The model under review builds one solid part; all positions refer to its coordinate system, in mm. Coordinates: 2 decimals unless noted, no trailing zeros. Order: outer loops, then holes, each group sorted by start corner. A loop starts at its lowest first (then second) coordinate and runs counter-clockwise, first axis right, second up. Notation, with made-up numbers: (75.5, -37) -> (118.5, -37) arc R15 cw to (118.5, -15) -> close; hole circle Ø6 at (-26.5, -36.5). An arc over 180 degrees is marked (long way). Put each result on its own line as item: value.
from build123d import *

# Parameters (mm, degrees)
SKETCH_1_R          = 4
EXTRUDE_1_DEPTH     = 105
CUT_EXTRUDE_1_DEPTH = 10
CUT_EXTRUDE_2_DEPTH = 59


with BuildPart() as part:
    # 草图1 → 凸台-拉伸1 (new body)
    with BuildSketch(Plane.XY):
        with Locations((-9.495904584, 0)):
            Circle(SKETCH_1_R)
    extrude(amount=EXTRUDE_1_DEPTH)

    # 草图2 → 切除-拉伸1 (cut)
    with BuildSketch(Plane(origin=(0, 0, 0), x_dir=(-1, 0, 0), z_dir=(0, 0, -1))):
        with BuildLine():
            Line((7.095904584, 3.2), (11.895904584, 3.2))
            ThreePointArc((11.895904584, 3.2), (9.495904584, 4), (7.095904584, 3.2))
        make_face()
    extrude(amount=-CUT_EXTRUDE_1_DEPTH, mode=Mode.SUBTRACT)

    # 草图3 → 切除-拉伸2 (cut)
    with BuildSketch(Plane(origin=(0, 0, 16), x_dir=(-1, 0, 0), z_dir=(0, 0, -1))):
        with BuildLine():
            Line((7.095904584, 3.2), (11.895904584, 3.2))
            ThreePointArc((11.895904584, 3.2), (9.495904584, 4), (7.095904584, 3.2))
        make_face()
    extrude(amount=-CUT_EXTRUDE_2_DEPTH, mode=Mode.SUBTRACT)


solid = part.part
Item 1: Consider section D-D on z = 85. Write out the cut boundary in (x, y).
Answers below:
outline: circle Ø8 at (-9.5, 0)
Item 2: Consider section B-B on z = 43. Write out the cut boundary in (x, y).
Answers below:
outline: (-11.9, 3.2) arc R4 ccw (long way) to (-7.1, 3.2) -> close
Item 3: For line 1 (Z direction, x = -11.75, y = 3.25); line 2 (X direction, y = 0.25, z = 72.5); line 3 (X direction, y = -3.5, z = 90.5), list the stretches that pass through material, from the lowest coordinate up. Write a range as from..to.
Answers below:
line 1: 10..16, 75..105
line 2: -13.49..-5.5
line 3: -11.43..-7.56
Item 4: Consider section A-A on x = -10.75. Write out the cut boundary in (y, z).
Answers below:
outline: (-3.8, 0) -> (3.2, 0) -> (3.2, 10) -> (3.8, 10) -> (3.8, 16) -> (3.2, 16) -> (3.2, 75) -> (3.8, 75) -> (3.8, 105) -> (-3.8, 105) -> close
Item 5: Consider section C-C on y = 1.75. Write out the cut boundary in (x, z).
Answers below:
outline: (-13.09, 0) -> (-5.9, 0) -> (-5.9, 105) -> (-13.09, 105) -> close
Item 6: Mouldability with a two-part tool opening along Z and no side actions: class faces 1 (the flat face through (-9, 3.2, 45)), 2 (the flat face through (-10, 0, 0)), 3 (the flat face through (-9, 3.2, 5)) as +Z half, -Z half, draft (parallel to the pull), parting line (faces both ways), or undercut.
Answers below:
face 1: undercut
face 2: -Z half
face 3: draft
Item 7: For pin 1 Ø1.5 at (x, y) = (-12, 1.5) entering from -Z; pin 2 Ø2 at (y, z) = (3, 73) entering from -X; pin 3 Ø2.5 at (x, z) = (-9, 5.5) entering from +Y; pin 4 Ø3 at (y, z) = (2.5, 11) entering from +X, all flat-tipped, find the tip position at first contact; note any pin that passes through.
Answers below:
pin 1: z = 0
pin 2: x = -12.96
pin 3: y = 3.2
pin 4: x = -5.62
